Could you check a few things on this drawing? It's one solid part, dimensions in mm from its lowest x, y, z. A direction names the side the tool comes from. Coordinates: 2 decimals unless noted, no trailing zeros. Write each loop counter-clockwise with the first axis right and the second up, starting at its lowest first coordinate (ties: lowest second). Pieces come first, ordered by that corner, then holes.
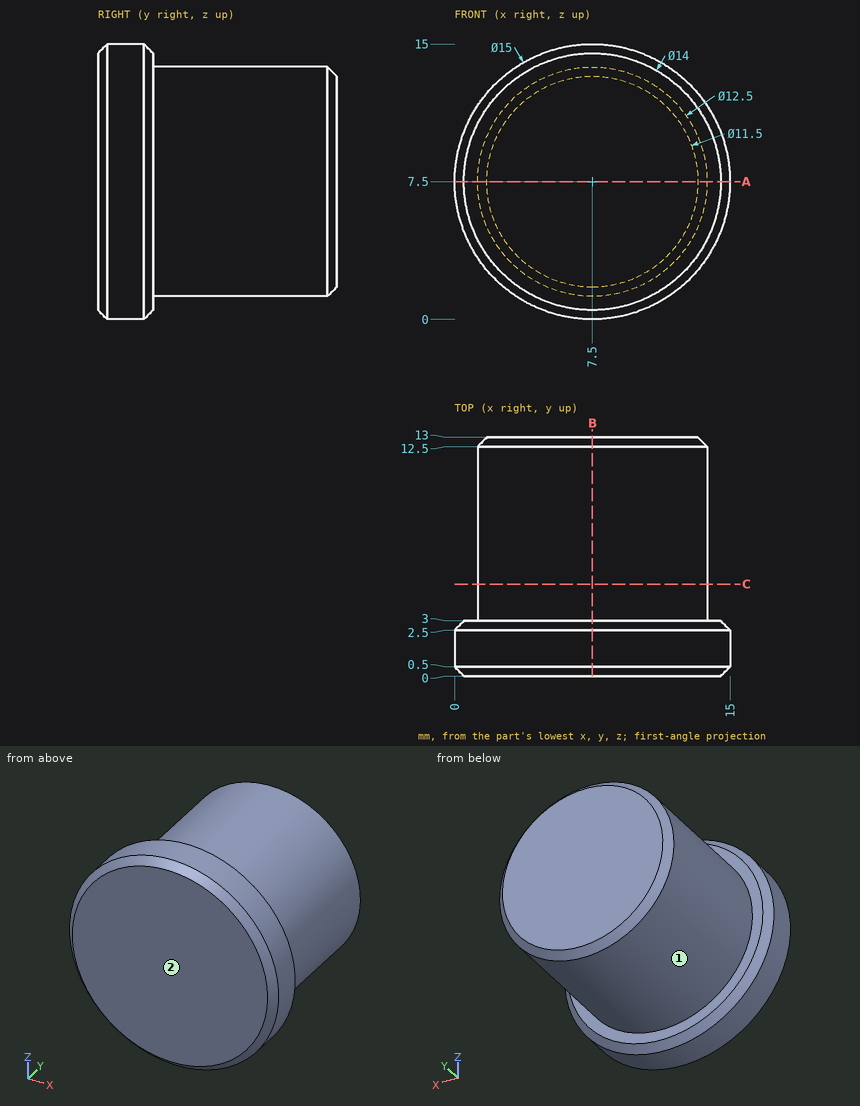
1) On a 3-axis mill with a long thin cutter (end or side, diameter ignored), from which of +Z, -Z, +X, -X, +Y, -Y can I reach the whole of each face in a straight line? I mean the marked faces 1 and 2. Say none if no direction works.
Values follow:
face 1: +Y
face 2: +Z, -Z, +X, -X, -Y
2) Will these pins go through, and if not, where does the flat tip stop? pin 1 (5 mm diameter, centred on x = 3, y = 10, fed in from +Z); pin 2 (3 mm diameter, centred on x = 4.5, y = 11.5, fed in from -Z); pin 3 (1 mm diameter, centred on x = 8, y = 6, fed in from +Z).
Values follow:
pin 1: stops at z = 13.42
pin 2: stops at z = 1.43
pin 3: stops at z = 13.75
3) Imagine slicing it at C-C on y = 5. Please give me the cut outline in (x, z), then the cut area to 3 significant figures.
Values follow:
outline: circle Ø12.5 at (7.5, 7.5)
area: 123 mm2
4) Imagine slicing it at B-B on x = 7.5. Please give me the cut outline in (y, z).
Values follow:
outline: (0, 0.5) - (0.5, 0) - (2.5, 0) - (3, 0.5) - (3, 1.25) - (12.5, 1.25) - (13, 1.75) - (13, 13.25) - (12.5, 13.75) - (3, 13.75) - (3, 14.5) - (2.5, 15) - (0.5, 15) - (0, 14.5) - close
5) I need wall thicknesses on probe 1 along X at (y, z) = (11.75, 7.5); probe 2 along Y at (x, z) = (4.5, 1.25); probe 3 along X at (y, z) = (10, 3.75). Which ranges of each line are inside material? Lowest first, please.
Values follow:
probe 1: x = 1.25 to 13.75
probe 2: y = 0 to 3
probe 3: x = 2.5 to 12.5
6) Imagine slicing it at A-A on z = 7.5. Please give me the cut outline in (x, y).
Values follow:
outline: (0, 0.5) - (0.5, 0) - (14.5, 0) - (15, 0.5) - (15, 2.5) - (14.5, 3) - (13.75, 3) - (13.75, 12.5) - (13.25, 13) - (1.75, 13) - (1.25, 12.5) - (1.25, 3) - (0.5, 3) - (0, 2.5) - close
